```python
from build123d import *

# Parameters (mm, degrees)
SKETCH1_W           = 43
SKETCH1_H           = 8
BOSS_EXTRUDE1_DEPTH = 2
SKETCH2_R           = 2.25
CUT_EXTRUDE1_DEPTH  = 35.195745727
SKETCH3_R           = 2
BOSS_EXTRUDE2_DEPTH = 1
CHAMFER2_SIZE       = 2


with BuildPart() as part:
    # Sketch1 → Boss-Extrude1 (new body)
    with BuildSketch(Plane(origin=(0, 0, 0), x_dir=(1, 0, 0), z_dir=(0, 1, 0))):
        with Locations((11.806648575, 3.484396201)):
            Rectangle(SKETCH1_W, SKETCH1_H)
    extrude(amount=BOSS_EXTRUDE1_DEPTH)

    # Sketch2 → Cut-Extrude1 (cut, through all)
    with BuildSketch(Plane(origin=(0, 2, 0), x_dir=(1, 0, 0), z_dir=(0, 1, 0))):
        with Locations(Location((-4.693351425, 3.484396201, 0), (0, 0, 270))):
            Circle(SKETCH2_R)
    extrude(amount=-CUT_EXTRUDE1_DEPTH, mode=Mode.SUBTRACT)

    # Sketch3 → Boss-Extrude2 (add)
    with BuildSketch(Plane(origin=(0, 2, 0), x_dir=(1, 0, 0), z_dir=(0, 1, 0))):
        with Locations(Location((29.306648575, 3.484396201, 0), (0, 0, 270))):
            Circle(SKETCH3_R)
    extrude(amount=BOSS_EXTRUDE2_DEPTH)

    # Chamfer2
    chamfer2_edges = [part.edges().sort_by_distance(p)[0] for p in [
        (-9.693351425, 1, -7.484396201),
        (33.306648575, 1, -7.484396201),
        (33.306648575, 1, 0.515603799),
        (-9.693351425, 1, 0.515603799),
    ]]
    chamfer(chamfer2_edges, length=CHAMFER2_SIZE)


solid = part.part
```
Input: part model. Units: mm. Frame: model coordinates. A direction names the side the tool comes from. Give positions to 0.01 mm unless a question says otherwise; leave off trailing zeros. Order: outer loops, then holes, each group sorted by start corner. A loop starts at its lowest first (then second) coordinate and runs counter-clockwise, first axis right, second up. Notation, with made-up numbers: M 82.25,22 L 87.25,22 A31 ccw 87.25,46 Z; hole C 31.5,33 d4. An arc over 180 degrees is marked long. One line per question, with ' | ' between items. Start each with the question number.
1. Section query A-A (z = -2). Return the cut outline in (x, y).
2. Section query D-D (z = -3.75). Return the cut outline in (x, y).
3. Section query C-C (y = 0.6). Return the cut outline in (x, z).
4. Material intervals for probe 1 along Y at (x, z) = (-6, -0.75); probe 2 along X at (y, z) = (0.9, -5.5); probe 3 along X at (y, z) = (1.35, -4), sorted ascending. Write a range as [from, to].
5. Pull-direction query (X, two-part tool) for faces 1 (the face through (-8.68, 0.99, -6.5)), 2 (the face through (-3.17, 1.01, -5.14)), 3 (the face through (12, 2, -4)); classes: released by +X, released by -X, zero draft, split by the parting line, or undercut.
6. Access query for faces 4 (the face through (-8.68, 0.99, -0.47)), 5 (the face through (27.354, 2.493, -3.918)). Directions: +Z, -Z, +X, -X, +Y, -Y. A direction counts if a zero-diameter tool reaches every point of the face in a straight line with its end or side. Return the directions, or none.
7. Section query B-B (x = -3.5). Return the cut outline in (y, z), and give its area (3 significant figures).
Here are the results:
1) outline: M -9.69,0 L -6.38,0 L -6.38,2 L -9.69,2 Z; M -3,0 L 33.31,0 L 33.31,2 L 30.65,2 L 30.65,3 L 27.97,3 L 27.97,2 L -3,2 Z
2) outline: M -9.69,0 L -6.93,0 L -6.93,2 L -9.69,2 Z; M -2.46,0 L 33.31,0 L 33.31,2 L 31.29,2 L 31.29,3 L 27.32,3 L 27.32,2 L -2.46,2 Z
3) outline: M -9.69,-5.48 L -7.69,-7.48 L 31.31,-7.48 L 33.31,-5.48 L 33.31,-1.48 L 31.31,0.52 L -7.69,0.52 L -9.69,-1.48 Z; hole C -4.69,-3.48 d4.5
4) probe 1: [0, 2] | probe 2: [-9.68, -5.69], [-3.69, 33.29] | probe 3: [-9.69, -6.88], [-2.5, 33.31]
5) face 1: released by -X | face 2: undercut | face 3: zero draft
6) face 4: +Z, -X, +Y, -Y | face 5: +Y
7) outline: M 0,-7.48 L 2,-7.48 L 2,-5.39 L 0,-5.39 Z; M 0,-1.58 L 2,-1.58 L 2,0.52 L 0,0.52 Z | area: 8.37 mm²
